Geometry: see drawing. Coordinates: mm, zero at the bounding-box minimum. Round coordinates to 2 decimals unless told otherwise and drop trailing zeros. Write each loop counter-clockwise with the first axis right and the second up, starting at its lowest first coordinate (ties: lowest second). Pieces come first, ordered by that corner, then holes.
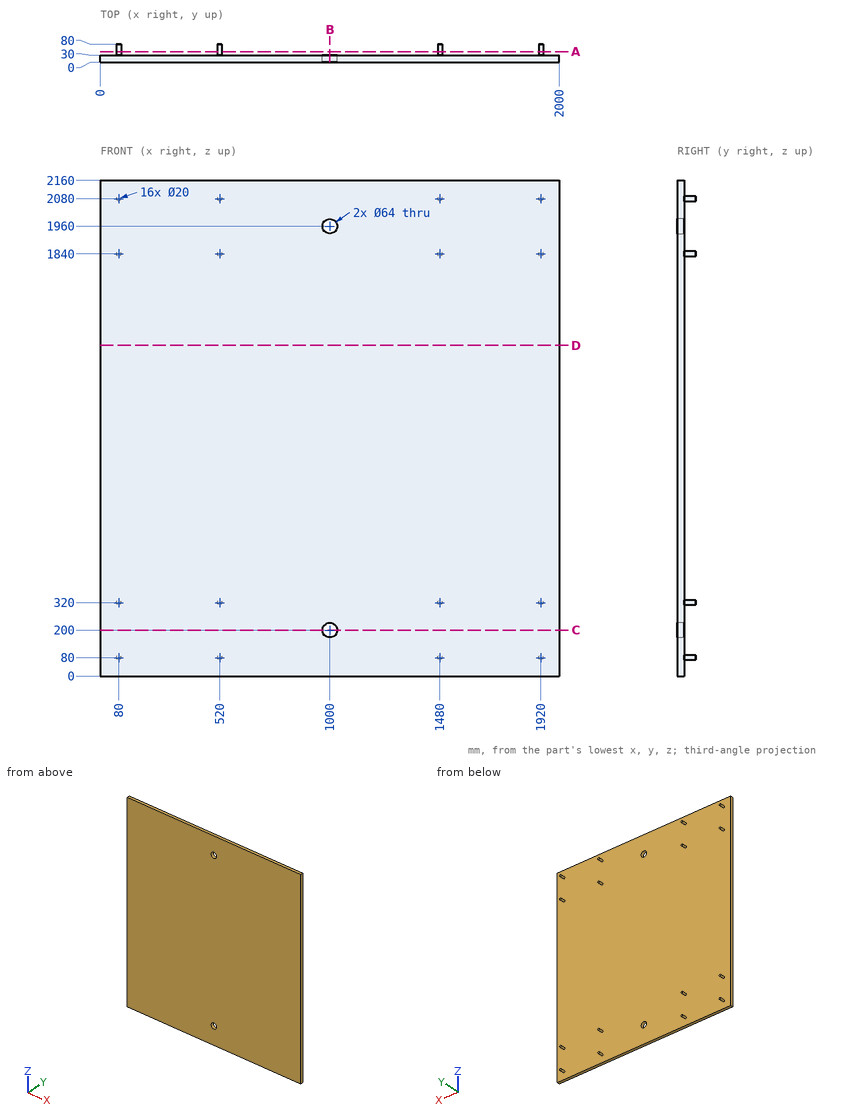
1) Section query D-D on z = 1440.5. Return the cut outline in (x, y).
Taken from the geometry:
outline: (0, 0) - (2000, 0) - (2000, 30) - (0, 30) - close
2) Section query A-A on y = 47. State how many separate pieces and enclosed holes the cut face has, then the cut area to 3 significant figures.
Taken from the geometry:
separate pieces: 16
enclosed holes: 0
area: 5,030 mm2
3) Section query B-B on x = 1000. Return the cut outline in (y, z), then the cut area to 3 significant figures.
Taken from the geometry:
outline: (0, 0) - (30, 0) - (30, 168) - (0, 168) - close; (0, 232) - (30, 232) - (30, 1928) - (0, 1928) - close; (0, 1992) - (30, 1992) - (30, 2160) - (0, 2160) - close
area: 61,000 mm2
4) Contact query for flat-ended pins moving along their axis: P1, Ø8, axis at x = 1445.5, z = 1048, coming from the -Y side; P2, Ø3, axis at x = 1177.5, z = 1688.5, coming from the +Y side. Output: stop coordinate, or through.
Taken from the geometry:
P1: stops at y = 0
P2: stops at y = 30
5) Section query C-C on z = 200. Return the cut outline in (x, y).
Taken from the geometry:
outline: (0, 0) - (968, 0) - (968, 30) - (0, 30) - close; (1032, 0) - (2000, 0) - (2000, 30) - (1032, 30) - close
6) Material intervals for line 1 (X direction, y = 66.5, z = 322.5); line 2 (X direction, y = 23, z = 200); line 3 (Y direction, x = 1812, z = 216.5), sorted ascending.
Taken from the geometry:
line 1: x = 70.32 to 89.68, 510.32 to 529.68, 1470.32 to 1489.68, 1910.32 to 1929.68
line 2: x = 0 to 968, 1032 to 2000
line 3: y = 0 to 30
